from build123d import *

# Parameters (mm, degrees)
EXTRUDE_1_DEPTH         = 10
HOLE_WIZARD_M12_1_D     = 10.2
HOLE_WIZARD_M12_1_DEPTH = 32.75
HOLE_WIZARD_M12_1_TIP   = 3.064389157


with BuildPart() as part:
    # 草图1 → 凸台-拉伸1 (new body)
    with BuildSketch(Plane.XY):
        Polygon((-30.845070423, -49.295774648), (-60.845070423, -19.295774648), (-60.845070423, 50.704225352), (59.154929577, 50.704225352), (59.154929577, -49.295774648), align=None)
    extrude(amount=EXTRUDE_1_DEPTH)

    # M12 螺纹孔1
    with Locations(Plane.XY.offset(10)):
        with Locations((9.154929577, 5.704225352)):
            Hole(HOLE_WIZARD_M12_1_D / 2, depth=HOLE_WIZARD_M12_1_DEPTH)
            with Locations((0, 0, -(HOLE_WIZARD_M12_1_DEPTH + HOLE_WIZARD_M12_1_TIP / 2))):  # 118° drill point
                Cone(0, HOLE_WIZARD_M12_1_D / 2, HOLE_WIZARD_M12_1_TIP, mode=Mode.SUBTRACT)


solid = part.part
Input: part model. Units: mm. Frame: model coordinates. Give positions to 0.01 mm unless a question says otherwise; leave off trailing zeros. Loops run counter-clockwise (first coordinate to the right, second up) from the corner with the lowest first, then second, coordinate; pieces in that order, holes last. Notation, with made-up numbers: M -38.5,68 L 7.5,68 A31 cw 7.5,105 Z; hole C -19.5,39 d10. An arc over 180 degrees is marked long. Use CSV: the item, a comma, the result in double quotes.
(1) Material intervals for L1, parallel to Y at x = 5.5, z = 3; L2, parallel to Y at x = 8, z = 4; L3, parallel to X at y = -33.5, z = 8.25, sorted ascending. Write a range as [from, to].
Outcome:
L1,"y = [-49.3, 2.15], [9.26, 50.7]"
L2,"y = [-49.3, 0.74], [10.67, 50.7]"
L3,"x = [-46.64, 59.15]"
(2) Section A-A, the plane y = 3.5. Return loops of the section in (x, z), plus the area to 3 significant figures.
Outcome:
outline,"M -60.85,0 L 4.56,0 L 4.56,10 L -60.85,10 Z; M 13.75,0 L 59.15,0 L 59.15,10 L 13.75,10 Z"
area,"1,110 mm²"
(3) Pull-direction query (X, two-part tool) for faces 1 (the face through (-60.845, 15, 5)), 2 (the face through (0, 1, 0)), 3 (the face through (13.2, 2.6, 4.9)); classes: pulls with the +X half, pulls with the -X half, needs draft (parallel to the pull), parting line crosses it, or undercut.
Outcome:
face 1,"pulls with the -X half"
face 2,"needs draft"
face 3,"undercut"
(4) Section B-B, the plane z = 1.75. Return loops of the section in (x, y).
Outcome:
outline,"M -60.85,-19.3 L -30.85,-49.3 L 59.15,-49.3 L 59.15,50.7 L -60.85,50.7 Z; hole C 9.15,5.7 d10.2"
